from build123d import *

# Parameters (mm, degrees)
SKETCH_1_R      = 442
EXTRUDE_1_DEPTH = 77.5


with BuildPart() as part:
    # 草图1 → 凸台-拉伸1 (new, symmetric)
    with BuildSketch(Plane.XY):
        Circle(SKETCH_1_R)
        Polygon((346.772490513, -23.298923219), (346.772490513, 23.298923219), (294.23960147, 184.978530989), (266.850074544, 222.676980659), (129.317185501, 322.600473549), (85, 337), (-85, 337), (-129.317185501, 322.600473549), (-266.850074544, 222.676980659), (-294.23960147, 184.978530989), (-346.772490513, 23.298923219), (-346.772490513, -23.298923219), (-294.23960147, -184.978530989), (-266.850074544, -222.676980659), (-129.317185501, -322.600473549), (-85, -337), (85, -337), (129.317185501, -322.600473549), (266.850074544, -222.67698066), (294.23960147, -184.978530989), align=None, mode=Mode.SUBTRACT)
    extrude(amount=EXTRUDE_1_DEPTH, both=True)


solid = part.part
Read the model definition and answer for the solid it produces. Units are mm, in the model's axes. A direction names the side the tool comes from. Give positions to 0.01 mm unless a question says otherwise; leave off trailing zeros. Write each loop counter-clockwise with the first axis right and the second up, starting at its lowest first coordinate (ties: lowest second). Pieces come first, ordered by that corner, then holes. Notation, with made-up numbers: M 18,-5.75 L 35,-5.75 A3 ccw 35,-1.75 Z; hole C 56,60 d4. An arc over 180 degrees is marked long. One line per item, written item: value. Start each with the question number.
(1) Find the intervals of material crossed by line 1 (Y direction, x = 5.5, z = -16); line 2 (Y direction, x = -12, z = -31); line 3 (X direction, y = -63.5, z = -33.5), in increasing order.
(2) Determine the mould class of faces 3 (the flat face through (325, 100, -77.5)), 4 (the flat face through (320.874, 103.007, 1.085)) for opening direction X: pulls with the +X half, pulls with the -X half, needs draft (parallel to the pull), parting line crosses it, or undercut.
(3) Find section C-C (z = -14.5). Determine the outline of the cut face in (x, y).
(4) Find section D-D (y = 375). Determine the outline of the cut face in (x, z), plus the area to 3 significant figures.
(5) Flat-ended cylindrical pins translate along their axes: pin 1 Ø4 at (y, z) = (102.5, -41) entering from +X; pin 2 Ø2 at (x, z) = (-58.5, 11.5) entering from +Y; pin 3 Ø10 at (y, z) = (218, 5) entering from -X. Find the tip coordinate at first contact, or state that the pin passes through.
(6) Find section A-A (y = 0). Determine the outline of the cut face in (x, z).
(7) Find section B-B (x = 0). Determine the outline of the cut face in (y, z), plus the area to 4 significant figures.
(8) A tool of negligible diameter and unlimited length cuts with its end or side. For faces 1 (the flat face through (325, 100, 77.5)), 2 (the flat face through (-106.85, 329.9, 1.09)), from which of +Z, -Z, +X, -X, +Y, -Y can it reach the whole face along a straight path? Write none if from no direction.
Results below:
1. line 1: y = -441.97 to -337, 337 to 441.97
1. line 2: y = -441.84 to -337, 337 to 441.84
1. line 3: x = -437.41 to -333.71, 333.71 to 437.41
2. face 3: needs draft
2. face 4: undercut
3. outline: C 0,0 d884; hole M -346.77,-23.3 L -294.24,-184.98 L -266.85,-222.68 L -129.32,-322.6 L -85,-337 L 85,-337 L 129.32,-322.6 L 266.85,-222.68 L 294.24,-184.98 L 346.77,-23.3 L 346.77,23.3 L 294.24,184.98 L 266.85,222.68 L 129.32,322.6 L 85,337 L -85,337 L -129.32,322.6 L -266.85,222.68 L -294.24,184.98 L -346.77,23.3 Z
4. outline: M -233.96,-77.5 L 233.96,-77.5 L 233.96,77.5 L -233.96,77.5 Z
4. area: 72,500 mm^2
5. pin 1: stops at x = 430.42
5. pin 2: stops at y = 438.24
5. pin 3: stops at x = -387.29
6. outline: M -442,-77.5 L -346.77,-77.5 L -346.77,77.5 L -442,77.5 Z; M 346.77,-77.5 L 442,-77.5 L 442,77.5 L 346.77,77.5 Z
7. outline: M -442,-77.5 L -337,-77.5 L -337,77.5 L -442,77.5 Z; M 337,-77.5 L 442,-77.5 L 442,77.5 L 337,77.5 Z
7. area: 32,550 mm^2
8. face 1: +Z, +X, -X, +Y, -Y
8. face 2: +Z, -Z
